from build123d import *

# Parameters (mm, degrees)
FORK_BODY_DEPTH                 = 35
LUG_CROSS_HOLE_SKETCH_R         = 6.5
LUG_CROSS_HOLE_13_DEPTH         = 105.763638969
BASE_MOUNTING_HOLES_SKETCH_R    = 6.5
BASE_MOUNTING_HOLES_2X_13_DEPTH = 84.312664103


with BuildPart() as part:
    # Fork Profile Sketch → Fork Body (new body)
    with BuildSketch(Plane.XY):
        Polygon((0, 0), (17.5, 0), (17.5, -19.374637846), (60, -19.374637846), (60, -5.374637846), (30, -5.374637846), (30, 40.625362154), (12.5, 40.625362154), (12.5, 14), (-12.5, 14), (-12.5, 40.625362154), (-30, 40.625362154), (-30, -5.374637846), (-60, -5.374637846), (-60, -19.374637846), (-17.5, -19.374637846), (-17.5, 0), align=None)
    extrude(amount=FORK_BODY_DEPTH)

    # Lug Cross Hole Sketch → Lug Cross Hole Ø13 (cut, through all)
    with BuildSketch(Plane.ZY.offset(30)):
        with Locations((17.5, 26.625362154)):
            Circle(LUG_CROSS_HOLE_SKETCH_R)
    extrude(amount=-LUG_CROSS_HOLE_13_DEPTH, mode=Mode.SUBTRACT)

    # Base Mounting Holes Sketch → Base Mounting Holes 2xØ13 (cut, through all)
    with BuildSketch(Plane(origin=(0, -5.374637846, 0), x_dir=(1, 0, 0), z_dir=(0, 1, 0))):
        with Locations(Location((46.423898933, -20, 0), (0, 0, 180))):
            Circle(BASE_MOUNTING_HOLES_SKETCH_R)
        with Locations((-46.423898933, -20)):
            Circle(BASE_MOUNTING_HOLES_SKETCH_R)
    extrude(amount=-BASE_MOUNTING_HOLES_2X_13_DEPTH, mode=Mode.SUBTRACT)


solid = part.part
Geometry: final body of the model. Coordinates: model frame, mm. A direction names the side the tool comes from. Round coordinates to 2 decimals unless told otherwise and drop trailing zeros. Loops run counter-clockwise (first coordinate to the right, second up) from the corner with the lowest first, then second, coordinate; pieces in that order, holes last. Notation, with made-up numbers: (1.25, 50.5) - (8.25, 50.5) arc R26 ccw to (8.25, 88.5) - close; hole circle Ø2 at (13, -39.75). An arc over 180 degrees is marked (long way). Write each question's results on one line, items separated by ' | '. Start each with the question number.
1) Mould query, pull axis Y, two halves, no side actions, for faces 4 (the face through (21.13, 31.02, 12.71)), 5 (the face through (-1, 4, 0)), 6 (the face through (45, -5.375, 13)), 7 (the face through (-21.37, 31.02, 12.71)). Classes: released by +Y, released by -Y, zero draft, split by the parting line, or undercut.
2) First-contact query: P1, Ø1, axis at y = 3.5, z = 31.5, coming from the -X side; P2, Ø7.5, axis at x = -3, z = 14.5, coming from the +Y side; P3, Ø10.5, axis at x = 46.42, z = 20, coming from the +Y side. Flat tips, straight axial feed; report the tip coordinate or a pass-through.
3) Cut plane A-A on z = 28. Return loops of the section in (x, y).
4) Cut plane C-C on x = 49. Return loops of the section in (y, z).
5) Access query for faces 1 (the face through (-17.5, -10, 17)), 2 (the face through (-45, -5.375, 13)), 3 (the face through (30, 17, 17)). Directions: +Z, -Z, +X, -X, +Y, -Y. A direction counts if a zero-diameter tool reaches every point of the face in a straight line with its end or side. Return the directions, or none.
6) Cut plane D-D on z = 17.5. Count the separate pieces of the cut face and the enclosed holes in it, then the cut area to 3 significant figures.
7) Line query: probe 1 along X at (y, z) = (-7, 20.5); probe 2 along X at (y, z) = (-2, 19); probe 3 along X at (y, z) = (33, 7.5). Output: solid intervals per line, ascending. Write a range as [from, to].
8) Cut plane B-B on y = -3.5. Return loops of the section in (x, z), then the cut area to 3 significant figures.
Verdict:
1) face 4: undercut | face 5: zero draft | face 6: released by +Y | face 7: undercut
2) P1: stops at x = -30 | P2: stops at y = 14 | P3: passes through
3) outline: (-60, -19.37) - (-17.5, -19.37) - (-17.5, 0) - (17.5, 0) - (17.5, -19.37) - (60, -19.37) - (60, -5.37) - (30, -5.37) - (30, 40.63) - (12.5, 40.63) - (12.5, 14) - (-12.5, 14) - (-12.5, 40.63) - (-30, 40.63) - (-30, -5.37) - (-60, -5.37) - close
4) outline: (-19.37, 0) - (-5.37, 0) - (-5.37, 14.03) - (-19.37, 14.03) - close; (-19.37, 25.97) - (-5.37, 25.97) - (-5.37, 35) - (-19.37, 35) - close
5) face 1: +Z, -Z, -Y | face 2: +Z, -Z, -X, +Y | face 3: +Z, -Z, +X, +Y
6) separate pieces: 5 | enclosed holes: 0 | area: 2,310 mm2
7) probe 1: x = [-60, -52.9], [-39.94, -17.5], [17.5, 39.94], [52.9, 60] | probe 2: x = [-30, -17.5], [17.5, 30] | probe 3: x = [-30, -12.5], [12.5, 30]
8) outline: (-30, 0) - (-17.5, 0) - (-17.5, 35) - (-30, 35) - close; (17.5, 0) - (30, 0) - (30, 35) - (17.5, 35) - close | area: 875 mm2
